Could you check a few things on this drawing? It's one solid part, dimensions in mm from its lowest x, y, z. Give positions to 0.01 mm unless a question says otherwise; leave off trailing zeros. Order: outer loops, then holes, each group sorted by start corner. A loop starts at its lowest first (then second) coordinate and runs counter-clockwise, first axis right, second up. Notation, with made-up numbers: M 59.5,35 L 73.5,35 A23 ccw 73.5,66 Z; hole C 13,64.25 d4. An arc over 180 degrees is marked long. Use one line per item in the form item = value.
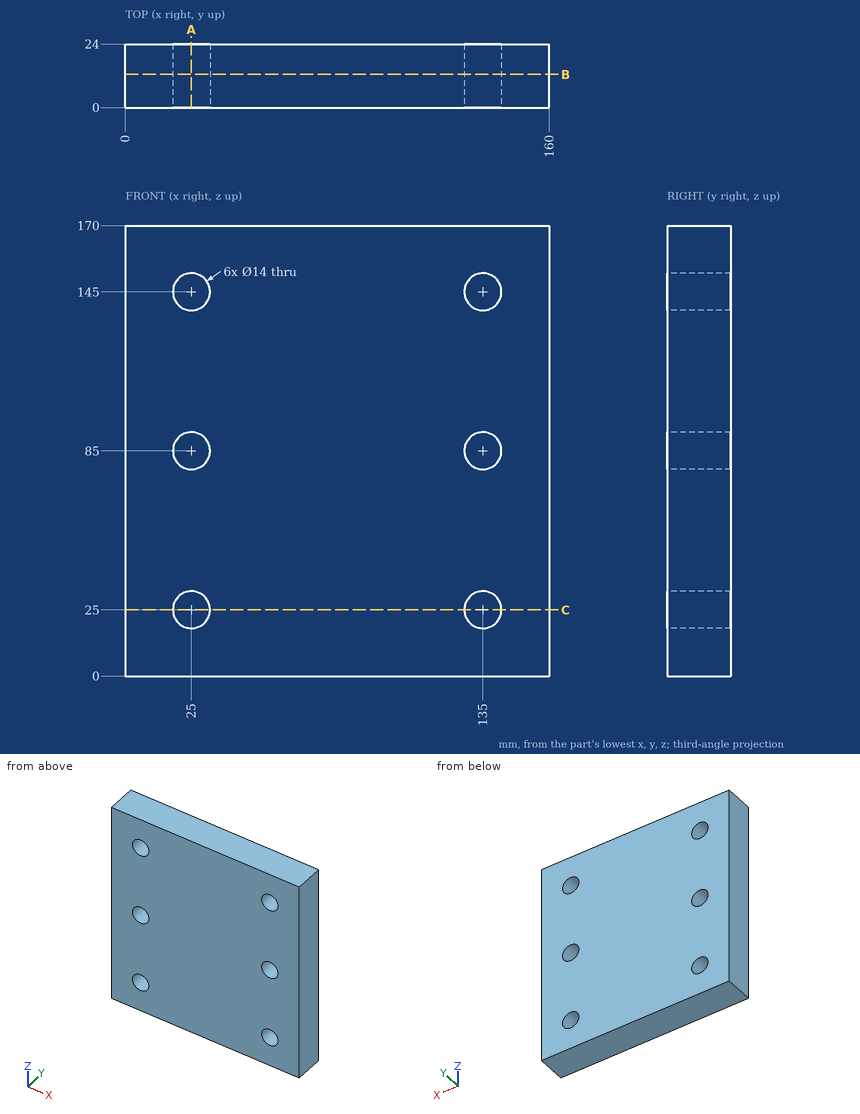
Q1. I want a section at C-C on z = 25. Write out the boundary of the cut face in (x, y), then the cut area to 3 significant figures.
Found:
outline = M 0,0 L 18,0 L 18,24 L 0,24 Z; M 32,0 L 128,0 L 128,24 L 32,24 Z; M 142,0 L 160,0 L 160,24 L 142,24 Z
area = 3,170 mm²
Q2. I want a section at A-A on x = 25. Write out the boundary of the cut face in (y, z).
Found:
outline = M 0,0 L 24,0 L 24,18 L 0,18 Z; M 0,32 L 24,32 L 24,78 L 0,78 Z; M 0,92 L 24,92 L 24,138 L 0,138 Z; M 0,152 L 24,152 L 24,170 L 0,170 Z
Q3. I need wall thicknesses on L1, parallel to X at y = 6, z = 145; L2, parallel to Z at x = 135, y = 17.5; L3, parallel to X at y = 21.25, z = 20. Which ranges of each line are inside material? Lowest first, please.
Found:
L1 = 0 to 18, 32 to 128, 142 to 160
L2 = 0 to 18, 32 to 78, 92 to 138, 152 to 170
L3 = 0 to 20.1, 29.9 to 130.1, 139.9 to 160
Q4. I want a section at B-B on y = 12.5. Write out the boundary of the cut face in (x, z), then the cut area to 3 significant figures.
Found:
outline = M 0,0 L 160,0 L 160,170 L 0,170 Z; hole C 25,25 d14; hole C 25,85 d14; hole C 25,145 d14; hole C 135,25 d14; hole C 135,85 d14; hole C 135,145 d14
area = 26,300 mm²
